Geometry check sheet. Reference: drawing and pictorial views, mm from the part's lowest x, y, z. Round coordinates to 2 decimals unless told otherwise and drop trailing zeros. Order: outer loops, then holes, each group sorted by start corner. A loop starts at its lowest first (then second) coordinate and runs counter-clockwise, first axis right, second up.
(1) Sectioned sample at A-A (z = 12.5). Record the boundary of the cut face in (x, y).
(2) Sectioned sample at C-C (y = 21). Record the boundary of the cut face in (x, z).
(3) Release check for a two-part mould opening along Z. For the marked faces 1, 2 and 3 record: +Z half, -Z half, draft (parallel to the pull), parting line (faces both ways), or undercut.
(4) Material ranges on line 1 along Z through (x, y) = (12.5, 12); line 2 along X through (y, z) = (14, 10.75); line 3 along X through (y, z) = (24.5, 8.5), recorded low to high.
(5) Sectioned sample at B-B (x = 12.5). Record the boundary of the cut face in (y, z), plus the area to 3 significant figures.
(6) Go/stop test with a flat-tipped pin: pin 1 (3 mm diameter, centred on x = 12, z = 10, fed in from -Y). Record where the tip stops, or that it passes through.
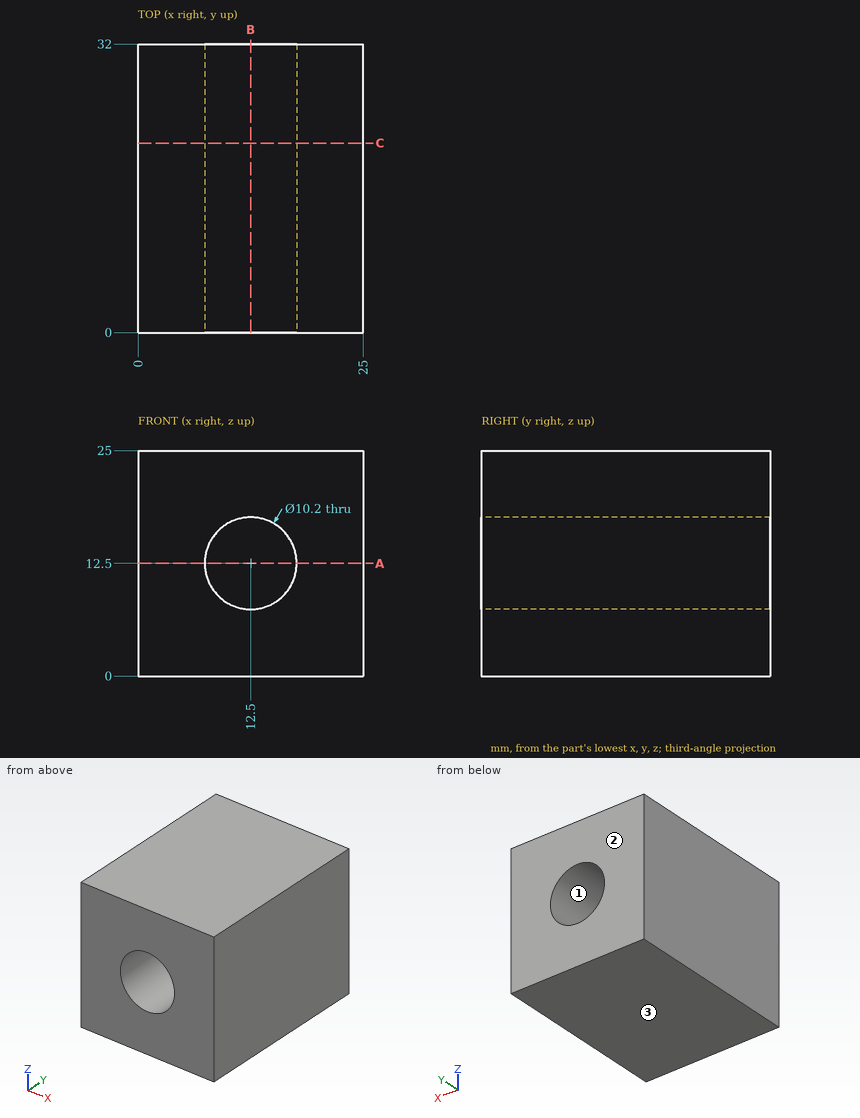
Answer below:
1. outline: (0, 0) - (7.4, 0) - (7.4, 32) - (0, 32) - close; (17.6, 0) - (25, 0) - (25, 32) - (17.6, 32) - close
2. outline: (0, 0) - (25, 0) - (25, 25) - (0, 25) - close; hole circle Ø10.2 at (12.5, 12.5)
3. face 1: undercut
3. face 2: draft
3. face 3: -Z half
4. line 1: z = 0 to 7.4, 17.6 to 25
4. line 2: x = 0 to 7.71, 17.29 to 25
4. line 3: x = 0 to 9.34, 15.66 to 25
5. outline: (0, 0) - (32, 0) - (32, 7.4) - (0, 7.4) - close; (0, 17.6) - (32, 17.6) - (32, 25) - (0, 25) - close
5. area: 474 mm2
6. pin 1: passes through
